Geometry check sheet. Reference: the model listing, model coordinates, mm. A direction names the side the tool comes from. Give positions to 0.01 mm unless a question says otherwise; leave off trailing zeros. Order: outer loops, then holes, each group sorted by start corner. A loop starts at its lowest first (then second) coordinate and runs counter-clockwise, first axis right, second up. Notation, with made-up numbers: (40.25, 30) - (87.25, 30) arc R16 ccw to (87.25, 55) - close; hole circle Ø7 at (46, 88.5). An arc over 180 degrees is marked (long way). Put each result on its own line as item: value. Start each with the question number.
```python
from build123d import *

# Parameters (mm, degrees)
SKETCH_1_R         = 32.5
SKETCH_1_R_2       = 23.5
EXTRUDE_1_DEPTH    = 3
SKETCH_2_R         = 32.5
SKETCH_2_R_2       = 25.5
EXTRUDE_2_DEPTH    = 4.8
HOLE_WIZARD_M4_1_D = 3.3


with BuildPart() as part:
    # 草图1 → 凸台-拉伸1 (new body)
    with BuildSketch(Plane(origin=(0, 0, 0), x_dir=(1, 0, 0), z_dir=(0, 1, 0))):
        with Locations(Location((0, 0, 0), (0, 0, 270))):
            Circle(SKETCH_1_R)
        with Locations(Location((0, 0, 0), (0, 0, 270))):
            Circle(SKETCH_1_R_2, mode=Mode.SUBTRACT)
    extrude(amount=EXTRUDE_1_DEPTH)

    # 草图2 → 凸台-拉伸2 (add)
    with BuildSketch(Plane(origin=(0, 3, 0), x_dir=(1, 0, 0), z_dir=(0, 1, 0))):
        with Locations(Location((0, 0, 0), (0, 0, 270))):
            Circle(SKETCH_2_R)
        with Locations(Location((0, 0, 0), (0, 0, 270))):
            Circle(SKETCH_2_R_2, mode=Mode.SUBTRACT)
    extrude(amount=EXTRUDE_2_DEPTH)

    # M4 螺纹孔1 (through all)
    with Locations(Plane(origin=(0, 7.8, 0), x_dir=(1, 0, 0), z_dir=(0, 1, 0))):
        with Locations((0, 29), (20.506096654, 20.506096654), (29, 0), (20.506096654, -20.506096654), (0, -29), (-20.506096654, -20.506096654), (-29, 0), (-20.506096654, 20.506096654), (0, 0)):
            Hole(HOLE_WIZARD_M4_1_D / 2)


solid = part.part
```
Item 1: Cross-section at D-D (x = 17.5). Enter the section's corners in (y, z).
Item 2: Thickness scan on line 1 along Z through (x, y) = (-0.5, 4); line 2 along Y through (x, z) = (24.5, 0); line 3 along X through (y, z) = (5, 13.5). Record the ranges inside material, lowest first.
Item 3: Cross-section at A-A (z = 0). Enter the section's corners in (x, y), and give its area (3 significant figures).
Item 4: Cross-section at C-C (y = 5). Count the separate pieces of the cut face and the enclosed holes in it, and give its area (3 significant figures).
Item 5: Set-up check for faces 1 (the face through (-21, 3, 11)), 2 (the face through (-20.29, 3.85, -22.14)): record each of +Z, -Z, +X, -X, +Y, -Y from which the full face is reachable in a straight line by a thin tool's end or side.
Item 6: Gauge pin test, flat ends, axial feed: pin 1 Ø1 at (x, z) = (21, -13.5) entering from +Y; pin 2 Ø2 at (y, z) = (5.5, 12) entering from +X; pin 3 Ø3 at (x, z) = (-20.51, 20.51) entering from -Y. Record the tip position at first contact, or that the pin passes through.
Item 7: Cross-section at B-B (x = 29). Enter the section's corners in (y, z), and give its area (3 significant figures).
Item 8: Release check for a two-part mould opening along X. For faces 3 (the face through (-22, 0, 9)), 4 (the face through (20.72, 3.85, 18.87)), 5 (the face through (9.76, 3.85, 31)) record: +X half, -X half, draft (parallel to the pull), parting line (faces both ways), or undercut.
Recorded:
1. outline: (0, -27.39) - (7.8, -27.39) - (7.8, -18.55) - (3, -18.55) - (3, -15.68) - (0, -15.68) - close; (0, 15.68) - (3, 15.68) - (3, 18.55) - (7.8, 18.55) - (7.8, 27.39) - (0, 27.39) - close
2. line 1: z = -32.5 to -30.57, -27.43 to -25.5, 25.5 to 27.43, 30.57 to 32.5
2. line 2: y = 0 to 3
2. line 3: x = -29.56 to -21.63, 21.63 to 29.56
3. outline: (-32.5, 0) - (-30.65, 0) - (-30.65, 7.8) - (-32.5, 7.8) - close; (-27.35, 0) - (-23.5, 0) - (-23.5, 3) - (-25.5, 3) - (-25.5, 7.8) - (-27.35, 7.8) - close; (23.5, 0) - (27.35, 0) - (27.35, 7.8) - (25.5, 7.8) - (25.5, 3) - (23.5, 3) - close; (30.65, 0) - (32.5, 0) - (32.5, 7.8) - (30.65, 7.8) - close
3. area: 69.7 mm^2
4. separate pieces: 1
4. enclosed holes: 9
4. area: 1,210 mm^2
5. face 1: +Y
5. face 2: +Y, -Y
6. pin 1: stops at y = 3
6. pin 2: stops at x = 30.58
6. pin 3: passes through
7. outline: (0, -14.67) - (7.8, -14.67) - (7.8, -1.65) - (0, -1.65) - close; (0, 1.65) - (7.8, 1.65) - (7.8, 14.67) - (0, 14.67) - close
7. area: 203 mm^2
8. face 3: draft
8. face 4: undercut
8. face 5: parting line
